Could you check a few things on this model? Use its own coordinates, in mm. A direction names the side the tool comes from. Coordinates: 2 decimals unless noted, no trailing zeros. Order: outer loops, then holes, each group sorted by start corner. A loop starts at its lowest first (then second) coordinate and runs counter-clockwise, first axis right, second up. Notation, with made-up numbers: (15, 72) - (66, 72) arc R10 ccw to (66, 88) - close; hole circle Ø4 at (51, 2.25). An arc over 180 degrees is marked (long way). One line per item, written item: value. Start each with the question number.
from build123d import *

# Parameters (mm, degrees)
SKETCH1_W                                         = 50
SKETCH1_H                                         = 220
BOSS_EXTRUDE1_DEPTH                               = 10
HOLE_SIZE_BY_SOCKET_HEAD_CAP_SCREW_TY_D           = 6.6
HOLE_SIZE_BY_SOCKET_HEAD_CAP_SCREW_TY_CBORE_D     = 11
HOLE_SIZE_BY_SOCKET_HEAD_CAP_SCREW_TY_CBORE_DEPTH = 6.8
M6_TAPPED_HOLE1_D                                 = 5
M6_TAPPED_HOLE1_DEPTH                             = 15
M6_TAPPED_HOLE1_TIP                               = 1.502151548


with BuildPart() as part:
    # Sketch1 → Boss-Extrude1 (new body)
    with BuildSketch(Plane(origin=(0, 0, 0), x_dir=(1, 0, 0), z_dir=(0, 1, 0))):
        Rectangle(SKETCH1_W, SKETCH1_H)
    extrude(amount=BOSS_EXTRUDE1_DEPTH)

    # Hole Size (% by) Socket Head Cap Screw Type1 (through all)
    with Locations(Plane(origin=(0, 0, 0), x_dir=(-1, 0, 0), z_dir=(0, -1, 0))):
        with Locations((0, -80), (0, 80), (0, 0)):
            CounterBoreHole(HOLE_SIZE_BY_SOCKET_HEAD_CAP_SCREW_TY_D / 2, HOLE_SIZE_BY_SOCKET_HEAD_CAP_SCREW_TY_CBORE_D / 2, HOLE_SIZE_BY_SOCKET_HEAD_CAP_SCREW_TY_CBORE_DEPTH)

    # M6 Tapped Hole1
    with Locations(Plane(origin=(0, 10, 0), x_dir=(1, 0, 0), z_dir=(0, 1, 0))):
        with Locations((-17.5, 40), (-17.5, -40), (17.5, 40), (17.5, -40)):
            Hole(M6_TAPPED_HOLE1_D / 2, depth=M6_TAPPED_HOLE1_DEPTH)
            with Locations((0, 0, -(M6_TAPPED_HOLE1_DEPTH + M6_TAPPED_HOLE1_TIP / 2))):  # 118° drill point
                Cone(0, M6_TAPPED_HOLE1_D / 2, M6_TAPPED_HOLE1_TIP, mode=Mode.SUBTRACT)


solid = part.part
Q1. We'd pull the mould along X, two halves only. Please class faces 3 (the cylindrical face through (1.19, 3.35, 5.37)), 4 (the flat face through (0, 5, 110)), 5 (the flat face through (25, 5, 2)), 6 (the cylindrical face through (19, 5, -38)): +X half, -X half, draft (parallel to the pull), parting line (faces both ways), or undercut.
Q2. If I drill on L1, parallel to Z at x = -17.5, y = 7.25; L2, parallel to X at y = 4.25, z = 40; L3, parallel to Z at x = 0, y = 5.5, over which ranges is the centre line in solid material (lowest first)?
Q3. I want a section at B-B on y = 8.5. Please give me the cut outline in (x, z).
Q4. I'm going to push a flat-ended pin straight in: pin 1 (5.5 mm diameter, centred on x = 0, z = -82.5, fed in from -Y). Where does the tip first touch, or does it pass through?
Q5. I want a section at D-D on x = 0. Please give me the cut outline in (y, z), then the cut area to 3 significant figures.
Q6. Which directions (+Z, -Z, +X, -X, +Y, -Y) give clear straight access to the entire face, cutting with the end or side of a thin tool? Please do faces 1 (the flat face through (0, 5, -110)), 2 (the cylindrical face through (0.716, 3.352, -85.453)).
Q7. I want a section at C-C on z = 0. Please give me the cut outline in (x, y).
Q8. I want a section at A-A on x = 17.5. Please give me the cut outline in (y, z), then the cut area to 3 significant figures.
Values follow:
1. face 3: undercut
1. face 4: draft
1. face 5: +X half
1. face 6: undercut
2. L1: z = -110 to -42.5, -37.5 to 37.5, 42.5 to 110
2. L2: x = -25 to -20, -15 to 15, 20 to 25
2. L3: z = -110 to -85.5, -74.5 to -5.5, 5.5 to 74.5, 85.5 to 110
3. outline: (-25, -110) - (25, -110) - (25, 110) - (-25, 110) - close; hole circle Ø5 at (-17.5, -40); hole circle Ø5 at (-17.5, 40); hole circle Ø6.6 at (0, -80); hole circle Ø6.6 at (0, 0); hole circle Ø6.6 at (0, 80); hole circle Ø5 at (17.5, -40); hole circle Ø5 at (17.5, 40)
4. pin 1: stops at y = 6.8
5. outline: (0, -110) - (10, -110) - (10, -83.3) - (6.8, -83.3) - (6.8, -85.5) - (0, -85.5) - close; (0, -74.5) - (6.8, -74.5) - (6.8, -76.7) - (10, -76.7) - (10, -3.3) - (6.8, -3.3) - (6.8, -5.5) - (0, -5.5) - close; (0, 5.5) - (6.8, 5.5) - (6.8, 3.3) - (10, 3.3) - (10, 76.7) - (6.8, 76.7) - (6.8, 74.5) - (0, 74.5) - close; (0, 85.5) - (6.8, 85.5) - (6.8, 83.3) - (10, 83.3) - (10, 110) - (0, 110) - close
5. area: 1,910 mm^2
6. face 1: -Z, +X, -X, +Y, -Y
6. face 2: -Y
7. outline: (-25, 0) - (-5.5, 0) - (-5.5, 6.8) - (-3.3, 6.8) - (-3.3, 10) - (-25, 10) - close; (3.3, 6.8) - (5.5, 6.8) - (5.5, 0) - (25, 0) - (25, 10) - (3.3, 10) - close
8. outline: (0, -110) - (10, -110) - (10, -42.5) - (0, -42.5) - close; (0, -37.5) - (10, -37.5) - (10, 37.5) - (0, 37.5) - close; (0, 42.5) - (10, 42.5) - (10, 110) - (0, 110) - close
8. area: 2,100 mm^2
